```python
from build123d import *

# Parameters (mm, degrees)
EXTRUDE_2_DEPTH          = 100
CUT_EXTRUDE_1_DEPTH      = 140.946373206
CUT_EXTRUDE_1_DEPTH_BACK = 140.946373206
SKETCH_2_W               = 5
SKETCH_2_H               = 42.071067812
EXTRUDE_3_DEPTH          = 10


with BuildPart() as part:
    # 草图1 → 凸台-拉伸2 (new body)
    with BuildSketch(Plane.XY):
        Polygon((0, 0), (0, -50), (40, -90), (43.535533906, -86.464466094), (5, -47.928932188), (5, 0), align=None)
    extrude(amount=EXTRUDE_2_DEPTH)

    # 草图2 → 切除-拉伸1 (cut, two sides: drawn at the far end of the back side and taken through both)
    with BuildSketch(Plane(origin=(5, 0, 0), x_dir=(0, 0, -1), z_dir=(1, 0, 0)).offset(-CUT_EXTRUDE_1_DEPTH_BACK)):
        Polygon((0, 0), (-5, 0), (-5, -5), (-5, -42.928932188), (-5, -47.928932188), (0, -47.928932188), align=None)
        with Locations((-2.5, -68.964466094)):
            Rectangle(SKETCH_2_W, SKETCH_2_H)
        with Locations((-97.5, -68.964466094)):
            Rectangle(SKETCH_2_W, SKETCH_2_H)
        Polygon((-95, -5), (-95, 0), (-100, 0), (-100, -47.928932188), (-95, -47.928932188), (-95, -42.928932188), align=None)
    extrude(amount=CUT_EXTRUDE_1_DEPTH + CUT_EXTRUDE_1_DEPTH_BACK, mode=Mode.SUBTRACT)

    # 草图3 → 凸台-拉伸3 (add)
    with BuildSketch(Plane.XY.offset(95)):
        Polygon((0, -50), (40, -90), (43.535533906, -86.464466094), (5, -47.928932188), (5, 0), (0, 0), align=None)
    extrude(amount=EXTRUDE_3_DEPTH)


solid = part.part
```
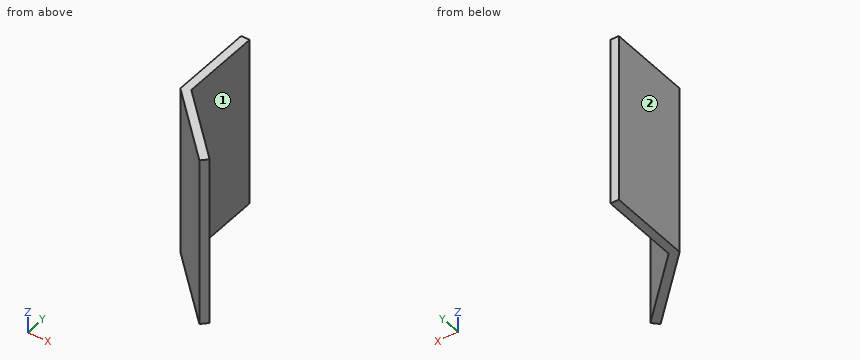
The model under review builds one solid part; all positions refer to its coordinate system, in mm. Face numbers are marked on the shaded views. A direction names the side the tool comes from. Give positions to 0.01 mm unless a question says otherwise; leave off trailing zeros. Write each loop counter-clockwise with the first axis right and the second up, starting at its lowest first coordinate (ties: lowest second). Pieces come first, ordered by that corner, then holes. Notation, with made-up numbers: M -24,-13.5 L -15,-13.5 A25 ccw -15,3.5 Z; hole C 86.25,88.5 d10. An arc over 180 degrees is marked long. Write item = value, one per line. Start each with the question number.
Q1. Clearance check with flat-ended pins moving along their axes: pin 1 (1.5 mm diameter, centred on x = 7, z = 67, fed in from +Y); pin 2 (4 mm diameter, centred on y = -11, z = 92.5, fed in from +X); pin 3 (1 mm diameter, centred on x = 16.5, z = 92, fed in from +Y). State where each tip first meets the part, or that it passes through.
Q2. We need section A-A (z = 31). State the section outline as (x, y) points.
Q3. Machinability: for the marked faces 1 and 2, which of the approach directions +Z, -Z, +X, -X, +Y, -Y give a long, thin tool a straight path to every point of the face, cutting with its end or side? Answer none if there is none.
Q4. We need section B-B (x = 3). State the section outline as (y, z) points, plus the area to 3 significant figures.
Q5. We need section C-C (y = -54). State the section outline as (x, z) points, plus the area to 3 significant figures.
Q6. For line 1 (X direction, y = -40.5, z = 100); line 2 (Y direction, x = 27.5, z = 23); line 3 (X direction, y = -77, z = 52), list the stretches that pass through material, from the lowest coordinate up.
Result set:
q1.pin_1 = -49.18
q1.pin_2 = 5
q1.pin_3 = -58.93
q2.outline = M 0,-50 L 40,-90 L 43.54,-86.46 L 5,-47.93 L 5,0 L 0,0 Z
q3.face_1 = +Z, -Z, +X, +Y
q3.face_2 = +Z, -Z, -X, +Y, -Y
q4.outline = M -53,5 L 0,5 L 0,105 L -53,105 Z
q4.area = 5,300 mm2
q5.outline = M 4,5 L 11.07,5 L 11.07,105 L 4,105 Z
q5.area = 707 mm2
q6.line_1 = 0 to 5
q6.line_2 = -77.5 to -70.43
q6.line_3 = 27 to 34.07
